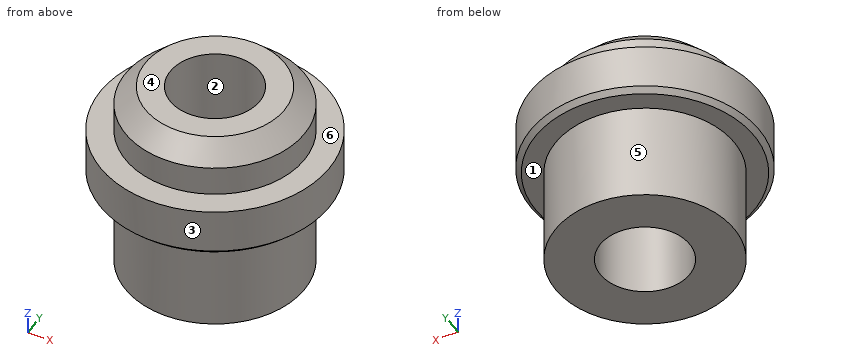
from build123d import *

# Parameters (mm, degrees)
SKETCH1_R           = 18
BOSS_EXTRUDE1_DEPTH = 20
SKETCH2_R           = 23
BOSS_EXTRUDE2_DEPTH = 10
SKETCH3_R           = 18
BOSS_EXTRUDE3_DEPTH = 10
CHAMFER1_SIZE       = 4
SKETCH4_R           = 9
CUT_EXTRUDE1_DEPTH  = 52.555795019
CHAMFER2_SIZE       = 1


with BuildPart() as part:
    # Sketch1 → Boss-Extrude1 (new body)
    with BuildSketch(Plane.XY):
        Circle(SKETCH1_R)
    extrude(amount=BOSS_EXTRUDE1_DEPTH)

    # Sketch2 → Boss-Extrude2 (add)
    with BuildSketch(Plane.XY.offset(20)):
        Circle(SKETCH2_R)
    extrude(amount=BOSS_EXTRUDE2_DEPTH)

    # Sketch3 → Boss-Extrude3 (add)
    with BuildSketch(Plane.XY.offset(30)):
        Circle(SKETCH3_R)
    extrude(amount=BOSS_EXTRUDE3_DEPTH)

    # Chamfer1
    chamfer1_edges = [part.edges().sort_by_distance(p)[0] for p in [
        (-18, 0, 40),
    ]]
    chamfer(chamfer1_edges, length=CHAMFER1_SIZE)

    # Sketch4 → Cut-Extrude1 (cut, through all)
    with BuildSketch(Plane.XY.offset(40)):
        Circle(SKETCH4_R)
    extrude(amount=-CUT_EXTRUDE1_DEPTH, mode=Mode.SUBTRACT)

    # Chamfer2
    chamfer2_edges = [part.edges().sort_by_distance(p)[0] for p in [
        (-23, 0, 20),
    ]]
    chamfer(chamfer2_edges, length=CHAMFER2_SIZE)


solid = part.part
Source: CAD feature listing. Evaluate the final solid. Frame: model axes, mm. Face numbers are marked on the shaded views. A direction names the side the tool comes from. Coordinates: 2 decimals unless noted, no trailing zeros. Order: outer loops, then holes, each group sorted by start corner. A loop starts at its lowest first (then second) coordinate and runs counter-clockwise, first axis right, second up. Notation, with made-up numbers: M 34.5,53 L 61.5,53 A25 cw 61.5,71 Z; hole C 31,62.25 d7. An arc over 180 degrees is marked long. Write each question's results on one line, items separated by ' | '. Start each with the question number.
1. Material intervals for L1, parallel to Y at x = 0, z = 25.5; L2, parallel to Y at x = 0, z = 31; L3, parallel to Z at x = -15, y = -14, sorted ascending.
2. Reachability of the marked faces 4, 5 and 6 from +Z, -Z, +X, -X, +Y, -Y: full face, straight path, thin tool, end or side. Return the list, or none.
3. Pin query (flat end, axial travel): pin 1 (6 mm diameter, centred on x = 13.5, z = 10.5, fed in from -Y); pin 2 (6 mm diameter, centred on y = -2, z = 16, fed in from +X); pin 3 (1 mm diameter, centred on x = -14.5, z = 5, fed in from +Y); pin 4 (1.5 mm diameter, centred on x = -3.5, y = 16.5, fed in from -Z). Return the tip coordinate at first contact, or that it passes through.
4. Section C-C, the plane z = 13. Return the cut outline in (x, y).
5. Draft query along Y for the marked faces 1, 2 and 3. Return one class per face: +Y half, -Y half, draft (parallel to the pull), parting line (faces both ways), or undercut.
6. Section D-D, the plane z = 37. Return the cut outline in (x, y).
7. Section A-A, the plane x = 0. Return the cut outline in (y, z), then the cut area to 3 significant figures.
Solution:
1) L1: -23 to -9, 9 to 23 | L2: -18 to -9, 9 to 18 | L3: 20 to 30
2) face 4: +Z, +X, -X, +Y, -Y | face 5: -Z | face 6: +Z
3) pin 1: y = -14.62 | pin 2: x = 18 | pin 3: y = 11.31 | pin 4: z = 0
4) outline: C 0,0 d36; hole C 0,0 d18
5) face 1: draft | face 2: undercut | face 3: parting line
6) outline: C 0,0 d34; hole C 0,0 d18
7) outline: M -23,21 L -22,20 L -18,20 L -18,0 L -9,0 L -9,40 L -14,40 L -18,36 L -18,30 L -23,30 Z; M 9,0 L 18,0 L 18,20 L 22,20 L 23,21 L 23,30 L 18,30 L 18,36 L 14,40 L 9,40 Z | area: 803 mm²
